Can you work these out from the model? Positions are in its coordinate system, mm. A direction names the side the tool comes from. Give positions to 0.01 mm unless a question says otherwise; leave off trailing zeros. Loops run counter-clockwise (first coordinate to the right, second up) from the corner with the lowest first, then second, coordinate; pieces in that order, holes last. Notation, with made-up numbers: (-9, 83.25) - (39, 83.25) arc R24 cw to (39, 106.25) - close; hole circle Ø9 at (66.25, 3). An arc over 180 degrees is marked (long way). Use a Markdown table: item, result. Add a question column.
```python
from build123d import *

# Parameters (mm, degrees)
SKETCH_1_W         = 45
SKETCH_1_H         = 165
EXTRUDE_1_DEPTH    = 125
SKETCH_3_W         = 45
SKETCH_3_H         = 32.5
EXTRUDE_2_DEPTH    = 2
HOLE_WIZARD_M4_1_D = 4.8
FILLET_1_R         = 5


with BuildPart() as part:
    # 草图1 → 凸台-拉伸1 (new body)
    with BuildSketch(Plane(origin=(0, 0, 0), x_dir=(1, 0, 0), z_dir=(0, 1, 0))):
        Rectangle(SKETCH_1_W, SKETCH_1_H)
    extrude(amount=EXTRUDE_1_DEPTH)

    # 草图3 → 凸台-拉伸2 (add)
    with BuildSketch(Plane(origin=(0, 0, 0), x_dir=(1, 0, 0), z_dir=(0, 1, 0))):
        with Locations((0, 98.75)):
            Rectangle(SKETCH_3_W, SKETCH_3_H)
        with Locations((0, -98.75)):
            Rectangle(SKETCH_3_W, SKETCH_3_H)
    extrude(amount=EXTRUDE_2_DEPTH)

    # M4 间隙孔1 (through all)
    with Locations(Plane(origin=(0, 2, 0), x_dir=(1, 0, 0), z_dir=(0, 1, 0))):
        with Locations((-15, 103), (15, 103), (15, -103), (-15, -103)):
            Hole(HOLE_WIZARD_M4_1_D / 2)

    # 圆角1
    fillet_1_edges = [part.edges().sort_by_distance(p)[0] for p in [
        (-22.5, 1, -115),
        (22.5, 1, -115),
        (-22.5, 1, 115),
        (22.5, 1, 115),
    ]]
    fillet(fillet_1_edges, radius=FILLET_1_R)


solid = part.part
```
1. Will these pins go through, and if not, where does the flat tip stop? P1, Ø5, axis at x = -4, y = 88, coming from the -Z side; P2, Ø10, axis at x = -1, z = -95.5, coming from the +Y side; P3, Ø10, axis at x = -10, y = 56.5, coming from the +Z side; P4, Ø3, axis at x = 15, z = 103, coming from the +Y side.
2. Suppose I cut it at B-B (z = 103). List the corners of the cut face in (x, y) for me, and give its area (3 significant figures).
3. Suppose I cut it at D-D (y = 116). List the corners of the cut face in (x, z) for me.
4. On a 3-axis mill with a long thin cutter (end or side, diameter ignored), from which of +Z, -Z, +X, -X, +Y, -Y can I reach the whole of each face in a straight line? I mean faces 4 (the face through (0, 2, -99)), 5 (the face through (-22.5, 62, 2)), 6 (the face through (0, 2, 99)). Say none if no direction works.
5. Suppose I cut it at A-A (x = -15). List the corners of the cut face in (y, z) for me, and give its area (3 significant figures).
6. Please list where these lines run through material, in increasing order: line 1 along Z through (x, y) = (-15, 1.2); line 2 along X through (y, z) = (1.15, 103); line 3 along Z through (x, y) = (15, 54). Write a range as [from, to].
7. Suppose I cut it at C-C (x = -0.5). List the corners of the cut face in (y, z) for me, and give its area (3 significant figures).
8. If we mould it in two halves opening along Z, with no side actions, what happens to faces 1 (the face through (15.31, 0.99, -105.38)), 2 (the face through (0, 63, 82.5)), 3 (the face through (0, 125, -1))? For each: released by +Z, released by -Z, zero draft, split by the parting line, or undercut.
Results below:
| question | item | result |
|---|---|---|
| 1 | P1 | z = -82.5 |
| 1 | P2 | y = 2 |
| 1 | P3 | z = 82.5 |
| 1 | P4 | through |
| 2 | outline | (-22.5, 0) - (-17.4, 0) - (-17.4, 2) - (-22.5, 2) - close; (-12.6, 0) - (12.6, 0) - (12.6, 2) - (-12.6, 2) - close; (17.4, 0) - (22.5, 0) - (22.5, 2) - (17.4, 2) - close |
| 2 | area | 70.8 mm² |
| 3 | outline | (-22.5, -82.5) - (22.5, -82.5) - (22.5, 82.5) - (-22.5, 82.5) - close |
| 4 | face 4 | -Z, +X, -X, +Y |
| 4 | face 5 | +Z, -Z, -X, +Y, -Y |
| 4 | face 6 | +Z, +X, -X, +Y |
| 5 | outline | (0, -115) - (2, -115) - (2, -105.4) - (0, -105.4) - close; (0, -100.6) - (2, -100.6) - (2, -82.5) - (125, -82.5) - (125, 82.5) - (2, 82.5) - (2, 100.6) - (0, 100.6) - close; (0, 105.4) - (2, 105.4) - (2, 115) - (0, 115) - close |
| 5 | area | 20,700 mm² |
| 6 | line 1 | [-115, -105.4], [-100.6, 100.6], [105.4, 115] |
| 6 | line 2 | [-22.5, -17.4], [-12.6, 12.6], [17.4, 22.5] |
| 6 | line 3 | [-82.5, 82.5] |
| 7 | outline | (0, -115) - (2, -115) - (2, -82.5) - (125, -82.5) - (125, 82.5) - (2, 82.5) - (2, 115) - (0, 115) - close |
| 7 | area | 20,800 mm² |
| 8 | face 1 | undercut |
| 8 | face 2 | released by +Z |
| 8 | face 3 | zero draft |
